For this review, take the finished solid that the model builds, in its own axes (mm). A direction names the side the tool comes from. Round coordinates to 2 decimals unless told otherwise and drop trailing zeros. Write each loop counter-clockwise with the first axis right and the second up, starting at its lowest first coordinate (ties: lowest second). Pieces come first, ordered by that corner, then holes.
from build123d import *

# Parameters (mm, degrees)
SKETCH1_W                    = 20
SKETCH1_H                    = 25
BOSS_EXTRUDE1_DEPTH          = 11
CHAMFER1_SIZE                = 2
M8_TAPPED_HOLE1_D            = 6.8
M4_TAPPED_HOLE1_D            = 3.3
M4_TAPPED_HOLE1_DEPTH        = 11.5
M4_TAPPED_HOLE1_TIP          = 0.991420021
F_4_0_4_DIAMETER_HOLE1_D     = 4
F_4_0_4_DIAMETER_HOLE1_DEPTH = 8
F_4_0_4_DIAMETER_HOLE1_TIP   = 1.201721238


with BuildPart() as part:
    # Sketch1 → Boss-Extrude1 (new, symmetric)
    with BuildSketch(Plane.XY):
        Rectangle(SKETCH1_W, SKETCH1_H)
    extrude(amount=BOSS_EXTRUDE1_DEPTH, both=True)

    # Chamfer1
    chamfer1_edges = [part.edges().sort_by_distance(p)[0] for p in [
        (-10, 12.5, 0),
        (10, 12.5, 0),
    ]]
    chamfer(chamfer1_edges, length=CHAMFER1_SIZE)

    # M8 Tapped Hole1 (through all)
    with Locations(Plane.XY.offset(11)):
        with Locations((0, 4)):
            Hole(M8_TAPPED_HOLE1_D / 2)

    # M4 Tapped Hole1
    with Locations(Plane(origin=(0, -12.5, 0), x_dir=(-1, 0, 0), z_dir=(0, -1, 0))):
        with Locations((6, -7), (-6, 7)):
            Hole(M4_TAPPED_HOLE1_D / 2, depth=M4_TAPPED_HOLE1_DEPTH)
            with Locations((0, 0, -(M4_TAPPED_HOLE1_DEPTH + M4_TAPPED_HOLE1_TIP / 2))):  # 118° drill point
                Cone(0, M4_TAPPED_HOLE1_D / 2, M4_TAPPED_HOLE1_TIP, mode=Mode.SUBTRACT)

    # Ø4.0 (4) Diameter Hole1
    with Locations(Plane(origin=(0, -12.5, 0), x_dir=(-1, 0, 0), z_dir=(0, -1, 0))):
        with Locations((-6, -7), (6, 7)):
            Hole(F_4_0_4_DIAMETER_HOLE1_D / 2, depth=F_4_0_4_DIAMETER_HOLE1_DEPTH)
            with Locations((0, 0, -(F_4_0_4_DIAMETER_HOLE1_DEPTH + F_4_0_4_DIAMETER_HOLE1_TIP / 2))):  # 118° drill point
                Cone(0, F_4_0_4_DIAMETER_HOLE1_D / 2, F_4_0_4_DIAMETER_HOLE1_TIP, mode=Mode.SUBTRACT)


solid = part.part
(1) Mouldability with a two-part tool opening along Z and no side actions: class faces 3 (the face through (4, -8, 7)), 4 (the face through (0, 0, 11)), 5 (the face through (9, 11.5, 0.2)), 6 (the face through (0, 0, -11)) as pulls with the +Z half, pulls with the -Z half, needs draft (parallel to the pull), parting line crosses it, or undercut.
Geometry check:
face 3: undercut
face 4: pulls with the +Z half
face 5: needs draft
face 6: pulls with the -Z half
(2) We need section C-C, the plane z = -3. Give the boundary of the cut face in (x, y), and give its area (3 significant figures).
Geometry check:
outline: (-10, -12.5) - (10, -12.5) - (10, 10.5) - (8, 12.5) - (-8, 12.5) - (-10, 10.5) - close; hole circle Ø6.8 at (0, 4)
area: 460 mm2
(3) For pin 1 Ø2.5 at (x, z) = (6, 7) entering from -Y, flat-tipped, find the tip position at first contact; note if it passes through.
Geometry check:
pin 1: stops at y = -4.05
(4) We need section A-A, the plane x = 0. Give the boundary of the cut face in (y, z).
Geometry check:
outline: (-12.5, -11) - (0.6, -11) - (0.6, 11) - (-12.5, 11) - close; (7.4, -11) - (12.5, -11) - (12.5, 11) - (7.4, 11) - close
(5) We need section D-D, the plane y = 2.25. Give the boundary of the cut face in (x, z), and give its area (3 significant figures).
Geometry check:
outline: (-10, -11) - (-2.92, -11) - (-2.92, 11) - (-10, 11) - close; (2.92, -11) - (10, -11) - (10, 11) - (2.92, 11) - close
area: 312 mm2
(6) We need section B-B, the plane y = -7.25. Give the boundary of the cut face in (x, z).
Geometry check:
outline: (-10, -11) - (10, -11) - (10, 11) - (-10, 11) - close; hole circle Ø4 at (-6, -7); hole circle Ø3.3 at (-6, 7); hole circle Ø4 at (6, 7); hole circle Ø3.3 at (6, -7)
(7) For line 1 along Z through (x, y) = (-6, -7.25); line 2 along Z through (x, y) = (6, -6.5); line 3 along X through (y, z) = (-2.5, -7), list the stretches that pass through material, from the lowest coordinate up.
Geometry check:
line 1: z = -11 to -9, -5 to 5.35, 8.65 to 11
line 2: z = -11 to -8.65, -5.35 to 5, 9 to 11
line 3: x = -10 to 4.35, 7.65 to 10
(8) For faces 1 (the face through (-6, -8, -9)), 2 (the face through (2.506, 6.298, -0.154)), list the 3-axis set-ups (+Z, -Z, +X, -X, +Y, -Y) from which the entire face can be reached by the end or side of a thin tool; tool diameter is ignored.
Geometry check:
face 1: -Y
face 2: +Z, -Z
